Geometry: final body of the model. Coordinates: model frame, mm. Face numbers are marked on the shaded views. Give positions to 0.01 mm unless a question says otherwise; leave off trailing zeros. Loops run counter-clockwise (first coordinate to the right, second up) from the corner with the lowest first, then second, coordinate; pieces in that order, holes last. Notation, with made-up numbers: (-12.5, -6) - (40.5, -6) arc R10 cw to (40.5, 0) - close; hole circle Ø7 at (-9.5, 30). An arc over 180 degrees is marked (long way). Use one line per item in the form item = value.
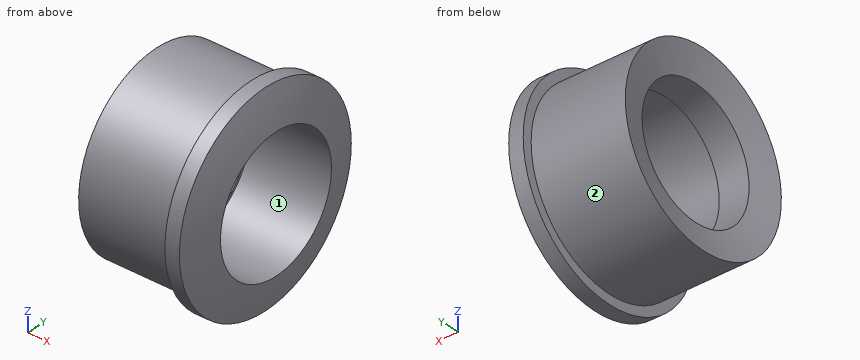
```python
from build123d import *

# Parameters (mm, degrees)
SKETCH3_R          = 20.25
CUT_EXTRUDE2_DEPTH = 12
SKETCH4_R          = 21
CUT_EXTRUDE3_DEPTH = 53.80624963


with BuildPart() as part:
    # Sketch1 → Revolve1 (revolve)
    with BuildSketch(Plane.XY):
        with BuildLine():
            Line((0, 0), (0, 29.5))
            Line((0, 29.5), (30, 29.5))
            Line((30, 29.5), (30, 32.5))
            Line((30, 32.5), (34.617976782, 32.5))
            ThreePointArc((34.617976782, 32.5), (36.49055142, 26.803395685), (38, 21))
            Line((38, 21), (38, 0))
            Line((38, 0), (0, 0))
        make_face()
    revolve(axis=Axis((38, 0, 0), (-1, 0, 0)))

    # Sketch3 → Cut-Extrude2 (cut)
    with BuildSketch(Plane.ZY):
        with Locations(Location((0, 0, 0), (0, 0, 270))):
            Circle(SKETCH3_R)
    extrude(amount=-CUT_EXTRUDE2_DEPTH, mode=Mode.SUBTRACT)

    # Cut-Extrude1 cone 1 section (through the dimple's axis) → Cut-Extrude1 (revolve, cut)
    with BuildSketch(Plane.ZX):
        Polygon((0, 0), (29.5, 0), (0, 7.904501177), align=None)
    revolve(axis=Axis((0, 0, 0), (1, 0, 0)), mode=Mode.SUBTRACT)

    # Sketch4 → Cut-Extrude3 (cut, through all)
    with BuildSketch(Plane.ZY.offset(-12)):
        with Locations(Location((0, 0, 0), (0, 0, 270))):
            Circle(SKETCH4_R)
    extrude(amount=-CUT_EXTRUDE3_DEPTH, mode=Mode.SUBTRACT)


solid = part.part
```
(1) Pull-direction query (Y, two-part tool) for the marked faces 1 and 2; classes: released by +Y, released by -Y, zero draft, split by the parting line, or undercut.
Solution:
face_1 = undercut
face_2 = split by the parting line
(2) Cut plane C-C (x = 18.5). Return the cut outline in (y, z), plus the area to 3 significant figures.
Solution:
outline = circle Ø59 at (0, 0); hole circle Ø42 at (0, 0)
area = 1,350 mm2
(3) Material intervals for L1, parallel to Z at x = 25.25, y = 0; L2, parallel to Y at x = 5, z = 0; L3, parallel to Y at x = 31.25, z = 0, sorted ascending. Write a range as from..to.
Solution:
L1 = -29.5..-21, 21..29.5
L2 = -29.5..-20.25, 20.25..29.5
L3 = -32.5..-21, 21..32.5
(4) Pin query (flat end, axial travel): P1, Ø12, axis at y = 8.5, z = -14, coming from the -X side; P2, Ø5, axis at x = 14.5, y = -15.5, coming from the +Z side; P3, Ø4, axis at x = 13.5, z = -15, coming from the -Y side. Return the tip coordinate at first contact, or that it passes through.
Solution:
P1 = 1.91
P2 = 26.48
P3 = -26.48
(5) Cut plane A-A (y = 0). Return the cut outline in (x, z).
Solution:
outline = (0, -29.5) - (30, -29.5) - (30, -32.5) - (34.62, -32.5) arc R95 ccw to (38, -21) - (12, -21) - (12, -20.25) - (2.48, -20.25) - close; (0, 29.5) - (2.48, 20.25) - (12, 20.25) - (12, 21) - (38, 21) arc R95 ccw to (34.62, 32.5) - (30, 32.5) - (30, 29.5) - close
